Input: part model. Units: mm. Frame: model coordinates. Face numbers are marked on the shaded views. A direction names the side the tool comes from. Round coordinates to 2 decimals unless told otherwise and drop trailing zeros. Order: outer loops, then holes, each group sorted by start corner. A loop starts at its lowest first (then second) coordinate and runs counter-clockwise, first axis right, second up.
Item 1: Cut plane D-D on z = 4.5. Output: boundary loops of the cut face in (x, y), then the cut area to 3 significant figures.
Item 2: First-contact query: pin 1 (15 mm diameter, centred on x = 23, z = 41, fed in from +Y); pin 2 (17 mm diameter, centred on y = 23, z = 22.5, fed in from -X); pin 3 (24 mm diameter, centred on x = 52.5, z = 39.5, fed in from +Y). Flat tips, straight axial feed; report the tip coordinate or a pass-through.
Item 3: Cut plane A-A on z = 39. Output: boundary loops of the cut face in (x, y), then the cut area to 3 significant figures.
Item 4: Line query: L1, parallel to Z at x = 50, y = 14; L2, parallel to Y at x = 66.5, z = 51; L3, parallel to X at y = 23.5, z = 17.5. Output: solid intervals per line, ascending.
Item 5: Reachability of the marked faces 1, 2 and 3 from +Z, -Z, +X, -X, +Y, -Y: full face, straight path, thin tool, end or side. Return the list, or none.
Item 6: Mould query, pull axis X, two halves, no side actions, for the marked faces 4, 5 and 6. Classes: released by +X, released by -X, zero draft, split by the parting line, or undercut.
Item 7: Cut plane C-C on y = 13. Output: boundary loops of the cut face in (x, z).
Item 8: Cut plane B-B on x = 60. Output: boundary loops of the cut face in (y, z), then the cut area to 3 significant figures.
```python
from build123d import *

# Parameters (mm, degrees)
BRACKET_BODY_DEPTH          = 12
CHAMFERED_PLATE_78X44_DEPTH = 10
CENTRE_PAD_SKETCH_W         = 30
CENTRE_PAD_SKETCH_H         = 50
CENTRE_PAD_30X30_DEPTH      = 6
PAD_POCKET_SKETCH_W         = 16
PAD_POCKET_SKETCH_H         = 16
PAD_POCKET_10X7_DEPTH       = 10
GUSSET_RIB_1_DEPTH          = 20
GUSSET_RIB_1_TRIM_DEPTH     = 10
GUSSET_RIB_2_DEPTH          = 20
GUSSET_RIB_2_TRIM_DEPTH     = 10


with BuildPart() as part:
    # Bracket Profile Sketch → Bracket Body (new body)
    with BuildSketch(Plane.XY):
        Polygon((3.579710145, 48), (3.579710145, 0), (93.579710145, 0), (93.579710145, 48), (81.579710145, 60), (15.579710145, 60), align=None)
    extrude(amount=BRACKET_BODY_DEPTH)

    # Chamfered Plate Sketch → Chamfered Plate 78x44 (add)
    with BuildSketch(Plane.XZ):
        Polygon((3.579710145, 12), (3.579710145, 56), (9.579710145, 62), (87.579710145, 62), (93.579710145, 56), (93.579710145, 12), align=None)
    extrude(amount=-CHAMFERED_PLATE_78X44_DEPTH)

    # Centre Pad Sketch → Centre Pad 30x30 (add)
    with BuildSketch(Plane(origin=(0, 10, 0), x_dir=(1, 0, 0), z_dir=(0, 1, 0))):
        with Locations((48.579710145, -37)):
            Rectangle(CENTRE_PAD_SKETCH_W, CENTRE_PAD_SKETCH_H)
    extrude(amount=CENTRE_PAD_30X30_DEPTH)

    # Pad Pocket Sketch → Pad Pocket 10x7 (cut)
    with BuildSketch(Plane(origin=(0, 16, 0), x_dir=(1, 0, 0), z_dir=(0, 1, 0))):
        with Locations((48.579710145, -30)):
            Rectangle(PAD_POCKET_SKETCH_W, PAD_POCKET_SKETCH_H)
    extrude(amount=-PAD_POCKET_10X7_DEPTH, mode=Mode.SUBTRACT)

    # Rib 1 Sketch → Gusset Rib 1 (add)
    with BuildSketch(Plane.ZY.offset(-3.579710145)):
        Polygon((12, 10), (12, 42), (33, 10), align=None)
    extrude(amount=-GUSSET_RIB_1_DEPTH)

    # Rib 1 Trim Sketch → Gusset Rib 1 Trim (cut)
    with BuildSketch(Plane.ZY.offset(-3.579710145)):
        Polygon((12, 42), (12, 10), (33, 10), align=None)
    extrude(amount=-GUSSET_RIB_1_TRIM_DEPTH, mode=Mode.SUBTRACT)

    # Rib 2 Sketch → Gusset Rib 2 (add)
    with BuildSketch(Plane(origin=(93.579710145, 0, 0), x_dir=(0, 0, -1), z_dir=(1, 0, 0))):
        Polygon((-12, 10), (-12, 42), (-33, 10), align=None)
    extrude(amount=-GUSSET_RIB_2_DEPTH)

    # Rib 2 Trim Sketch → Gusset Rib 2 Trim (cut)
    with BuildSketch(Plane(origin=(93.579710145, 0, 0), x_dir=(0, 0, -1), z_dir=(1, 0, 0))):
        Polygon((-12, 42), (-12, 10), (-33, 10), align=None)
    extrude(amount=-GUSSET_RIB_2_TRIM_DEPTH, mode=Mode.SUBTRACT)


solid = part.part
```
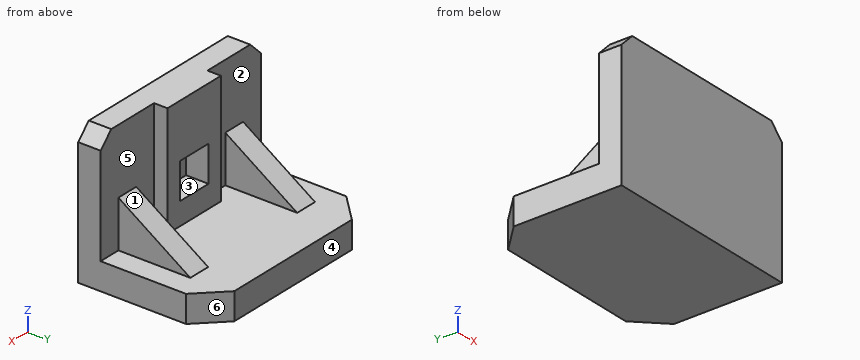
From the geometry:
1. outline: (3.58, 0) - (93.58, 0) - (93.58, 48) - (81.58, 60) - (15.58, 60) - (3.58, 48) - close
1. area: 5,260 mm2
2. pin 1: stops at y = 10
2. pin 2: stops at x = 13.58
2. pin 3: stops at y = 16
3. outline: (3.58, 0) - (93.58, 0) - (93.58, 10) - (63.58, 10) - (63.58, 16) - (33.58, 16) - (33.58, 10) - (3.58, 10) - close
3. area: 1,080 mm2
4. L1: z = 0 to 22, 38 to 62
4. L2: y = 0 to 10
4. L3: x = 13.58 to 23.58, 73.58 to 83.58
5. face 1: +Z, +X, +Y
5. face 2: +Z, +Y
5. face 3: +Y
6. face 4: zero draft
6. face 5: undercut
6. face 6: released by +X
7. outline: (3.58, 0) - (93.58, 0) - (93.58, 12) - (83.58, 12) - (83.58, 31.03) - (73.58, 31.03) - (73.58, 12) - (63.58, 12) - (63.58, 62) - (33.58, 62) - (33.58, 12) - (23.58, 12) - (23.58, 31.03) - (13.58, 31.03) - (13.58, 12) - (3.58, 12) - close; hole (40.58, 22) - (56.58, 22) - (56.58, 38) - (40.58, 38) - close
8. outline: (0, 0) - (60, 0) - (60, 12) - (16, 12) - (16, 62) - (0, 62) - close
8. area: 1,520 mm2
